Source: CAD feature listing. Evaluate the final solid. Frame: model axes, mm. Give positions to 0.01 mm unless a question says otherwise; leave off trailing zeros. Order: outer loops, then holes, each group sorted by start corner. A loop starts at its lowest first (then second) coordinate and runs counter-clockwise, first axis right, second up.
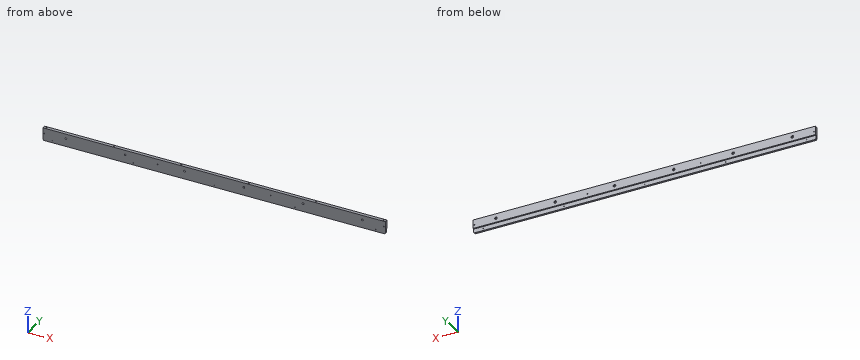
```python
from build123d import *

# Parameters (mm, degrees)
SKETCH_1_W             = 1270
SKETCH_1_H             = 47
EXTRUDE_1_DEPTH        = 6
SKETCH_2_W             = 15
SKETCH_2_H             = 5
CUT_EXTRUDE_1_DEPTH    = 1271.231573376
CHAMFER_1_SIZE         = 3
HOLE_WIZARD_M5_1_D     = 4.2
HOLE_WIZARD_M5_1_DEPTH = 12.4
HOLE_WIZARD_M5_1_TIP   = 1.2618073
HOLE_WIZARD_M4_1_D     = 3.3
HOLE_WIZARD_M3_1_D     = 2.5
HOLE_WIZARD_M8_1_D     = 6.8
SKETCH_12_R            = 5
CUT_EXTRUDE_2_DEPTH    = 3


with BuildPart() as part:
    # 草图1 → 凸台-拉伸1 (new, symmetric)
    with BuildSketch(Plane(origin=(0, 0, 0), x_dir=(1, 0, 0), z_dir=(0, 1, 0))):
        Rectangle(SKETCH_1_W, SKETCH_1_H)
    extrude(amount=EXTRUDE_1_DEPTH, both=True)

    # 草图2 → 切除-拉伸1 (cut, through all)
    with BuildSketch(Plane(origin=(635, 0, 0), x_dir=(0, 0, -1), z_dir=(1, 0, 0))):
        with Locations((16, 3.5)):
            Rectangle(SKETCH_2_W, SKETCH_2_H)
    extrude(amount=-CUT_EXTRUDE_1_DEPTH, mode=Mode.SUBTRACT)

    # 倒角1
    chamfer_1_edges = [part.edges().sort_by_distance(p)[0] for p in [
        (-635, -2.5, -23.5),
        (635, -2.5, -23.5),
    ]]
    chamfer(chamfer_1_edges, length=CHAMFER_1_SIZE)

    # M5 螺纹孔1
    with Locations(Plane.XY.offset(23.5)):
        with Locations((-625, 0), (-375, 0), (-125, 0), (125, 0), (375, 0), (625, 0)):
            Hole(HOLE_WIZARD_M5_1_D / 2, depth=HOLE_WIZARD_M5_1_DEPTH)
            with Locations((0, 0, -(HOLE_WIZARD_M5_1_DEPTH + HOLE_WIZARD_M5_1_TIP / 2))):  # 118° drill point
                Cone(0, HOLE_WIZARD_M5_1_D / 2, HOLE_WIZARD_M5_1_TIP, mode=Mode.SUBTRACT)

    # M4 螺纹孔1 (through all)
    with Locations(Plane(origin=(0, 6, 0), x_dir=(1, 0, 0), z_dir=(0, 1, 0))):
        with Locations((630, -3.5), (-630, -3.5), (210, -3.5), (-210, -3.5)):
            Hole(HOLE_WIZARD_M4_1_D / 2)

    # M3 螺纹孔1 (through all)
    with Locations(Plane(origin=(0, -6, 0), x_dir=(-1, 0, 0), z_dir=(0, -1, 0))):
        with Locations((-600, 16), (-300, 16), (0, 16), (300, 16), (600, 16)):
            Hole(HOLE_WIZARD_M3_1_D / 2)

    # M8 螺纹孔1 (through all)
    with Locations(Plane.XZ.offset(6)):
        with Locations((550, 6.5), (330, 6.5), (110, 6.5), (-110, 6.5), (-330, 6.5), (-550, 6.5)):
            Hole(HOLE_WIZARD_M8_1_D / 2)

    # 草图12 → 切除-拉伸2 (cut)
    with BuildSketch(Plane(origin=(0, 6, 0), x_dir=(1, 0, 0), z_dir=(0, 1, 0))):
        with Locations(Location((550, -6.5, 0), (0, 0, 270))):
            Circle(SKETCH_12_R)
        with Locations(Location((330, -6.5, 0), (0, 0, 270))):
            Circle(SKETCH_12_R)
        with Locations(Location((110, -6.5, 0), (0, 0, 270))):
            Circle(SKETCH_12_R)
        with Locations(Location((-110, -6.5, 0), (0, 0, 270))):
            Circle(SKETCH_12_R)
        with Locations(Location((-330, -6.5, 0), (0, 0, 270))):
            Circle(SKETCH_12_R)
        with Locations(Location((-550, -6.5, 0), (0, 0, 270))):
            Circle(SKETCH_12_R)
    extrude(amount=-CUT_EXTRUDE_2_DEPTH, mode=Mode.SUBTRACT)


solid = part.part
```
1) Pin query (flat end, axial travel): pin 1 (8 mm diameter, centred on x = 550, z = 6.5, fed in from +Y); pin 2 (5.5 mm diameter, centred on x = -309.5, y = 4.5, fed in from -Z); pin 3 (4 mm diameter, centred on x = 625, y = 0, fed in from +Z). Return the tip coordinate at first contact, or that it passes through.
Report:
pin 1: stops at y = 3
pin 2: stops at z = -8.5
pin 3: stops at z = 11.04
2) Material intervals for L1, parallel to X at y = -3, z = -16; L2, parallel to X at y = -5, z = 2.5; L3, parallel to Y at x = -388, z = -11.5, sorted ascending.
Report:
L1: x = -635 to -601.25, -598.75 to -301.25, -298.75 to -1.25, 1.25 to 298.75, 301.25 to 598.75, 601.25 to 635
L2: x = -635 to -631.31, -628.69 to -211.31, -208.69 to 208.69, 211.31 to 628.69, 631.31 to 635
L3: y = -6 to 1
3) Section query A-A, the plane x = 480.5. Return the cut outline in (y, z).
Report:
outline: (-6, -23.5) - (1, -23.5) - (1, -8.5) - (6, -8.5) - (6, 23.5) - (-6, 23.5) - close
